Geometry: final body of the model. Coordinates: model frame, mm. Face numbers are marked on the shaded views. A direction names the side the tool comes from. Give positions to 0.01 mm unless a question says otherwise; leave off trailing zeros. Order: outer loops, then holes, each group sorted by start corner. A loop starts at its lowest first (then second) coordinate and runs counter-clockwise, first axis right, second up. Notation, with made-up numbers: (68, -16) - (84, -16) arc R27 cw to (84, 22) - close; hole circle Ø2 at (30, 26.5). An arc over 180 degrees is marked (long way). Use one line per item in the form item = value.
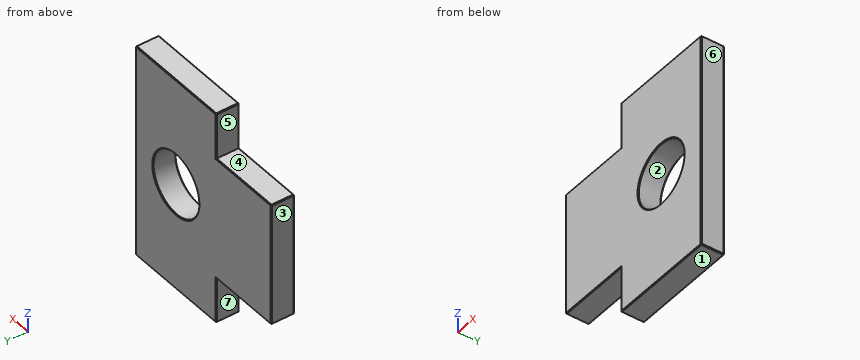
from build123d import *

# Parameters (mm, degrees)
SKETCH_1_R      = 20
EXTRUDE_1_DEPTH = 15
CHAMFER_1_SIZE  = 0.5


with BuildPart() as part:
    # 草图1 → 凸台-拉伸1 (new body)
    with BuildSketch(Plane(origin=(0, 0, 0), x_dir=(1, 0, 0), z_dir=(0, 1, 0))):
        Polygon((0, 70), (0, -70), (-70, -70), (-70, -40), (-118, -40), (-118, 40), (-70, 40), (-70, 70), align=None)
        with Locations(Location((-35, 0, 0), (0, 0, 270))):
            Circle(SKETCH_1_R, mode=Mode.SUBTRACT)
    extrude(amount=EXTRUDE_1_DEPTH)

    # 倒角1
    chamfer_1_edges = [part.edges().sort_by_distance(p)[0] for p in [
        (-35, 15, -70),
        (0, 0, 0),
        (-35, 0, 70),
        (-70, 15, -55),
        (-70, 7.5, 70),
        (-118, 7.5, 40),
        (-118, 7.5, -40),
        (-70, 7.5, -70),
        (0, 7.5, -70),
        (0, 7.5, 70),
        (-94, 15, -40),
        (-118, 15, 0),
        (-35, 0, -20),
        (-35, 15, -20),
        (-94, 15, 40),
        (-70, 15, 55),
        (-35, 15, 70),
        (0, 15, 0),
        (-70, 0, 55),
        (-94, 0, 40),
        (-118, 0, 0),
        (-94, 0, -40),
        (-70, 0, -55),
        (-35, 0, -70),
    ]]
    chamfer(chamfer_1_edges, length=CHAMFER_1_SIZE)


solid = part.part
(1) Cut plane B-B on y = 3. Output: boundary loops of the cut face in (x, z).
Computed values:
outline = (-118, -39.5) - (-117.5, -40) - (-70, -40) - (-70, -69.5) - (-69.5, -70) - (-0.5, -70) - (0, -69.5) - (0, 69.5) - (-0.5, 70) - (-69.5, 70) - (-70, 69.5) - (-70, 40) - (-117.5, 40) - (-118, 39.5) - close; hole circle Ø40 at (-35, 0)
(2) Contact query for a flat-ended pin moving along its axis: pin 1 Ø7 at (x, y) = (-104.5, 9.5) entering from +Z. Output: stop coordinate, or through.
Computed values:
pin_1 = 40
(3) Cut plane C-C on x = -35. Output: boundary loops of the cut face in (y, z), plus the area to 3 significant figures.
Computed values:
outline = (0, -69.5) - (0.5, -70) - (14.5, -70) - (15, -69.5) - (15, -20.5) - (14.5, -20) - (0.5, -20) - (0, -20.5) - close; (0, 20.5) - (0.5, 20) - (14.5, 20) - (15, 20.5) - (15, 69.5) - (14.5, 70) - (0.5, 70) - (0, 69.5) - close
area = 1,500 mm²
(4) Pull-direction query (Z, two-part tool) for the marked faces 1, 2, 3 and 4; classes: released by +Z, released by -Z, zero draft, split by the parting line, or undercut.
Computed values:
face_1 = released by -Z
face_2 = undercut
face_3 = zero draft
face_4 = released by +Z
(5) Ray query, line 1 along X through (y, z) = (9.25, 0); line 2 along Z through (x, y) = (-36, 12.5); line 3 along Z through (x, y) = (-104, 13.25). Return the intervals inside material, ascending.
Computed values:
line_1 = -118 to -55, -15 to 0
line_2 = -70 to -19.97, 19.97 to 70
line_3 = -40 to 40
(6) Cut plane D-D on x = -96.5. Output: boundary loops of the cut face in (y, z).
Computed values:
outline = (0, -39.5) - (0.5, -40) - (14.5, -40) - (15, -39.5) - (15, 39.5) - (14.5, 40) - (0.5, 40) - (0, 39.5) - close
(7) Reachability of the marked faces 5, 6 and 7 from +Z, -Z, +X, -X, +Y, -Y: full face, straight path, thin tool, end or side. Return the list, or none.
Computed values:
face_5 = +Z, -X, +Y, -Y
face_6 = +Z, -Z, +X, +Y, -Y
face_7 = -Z, -X, +Y, -Y
(8) Cut plane A-A on z = 0. Output: boundary loops of the cut face in (x, y).
Computed values:
outline = (-118, 0.5) - (-117.5, 0) - (-55.5, 0) - (-55, 0.5) - (-55, 14.5) - (-55.5, 15) - (-117.5, 15) - (-118, 14.5) - close; (-15, 0.5) - (-14.5, 0) - (-0.5, 0) - (0, 0.5) - (0, 14.5) - (-0.5, 15) - (-14.5, 15) - (-15, 14.5) - close
